The listing builds one solid part. Answer for the finished solid, in the listing's coordinates (mm). Face numbers are marked on the shaded views. Give positions to 0.01 mm unless a question says otherwise; leave off trailing zeros. Write each loop counter-clockwise with the first axis right and the second up, starting at its lowest first coordinate (ties: lowest second). Pieces come first, ordered by that corner, then holes.
```python
from build123d import *

# Parameters (mm, degrees)
SKETCH_1_R      = 5.1
EXTRUDE_1_DEPTH = 12


with BuildPart() as part:
    # 草图1 → 凸台-拉伸1 (new, symmetric)
    with BuildSketch(Plane.XY):
        with BuildLine():
            Line((0, 15), (30, 15))
            Line((30, 15), (30, -15))
            Line((30, -15), (0, -15))
            ThreePointArc((0, -15), (-15, 0), (0, 15))
        make_face()
        Circle(SKETCH_1_R, mode=Mode.SUBTRACT)
    extrude(amount=EXTRUDE_1_DEPTH, both=True)


solid = part.part
```
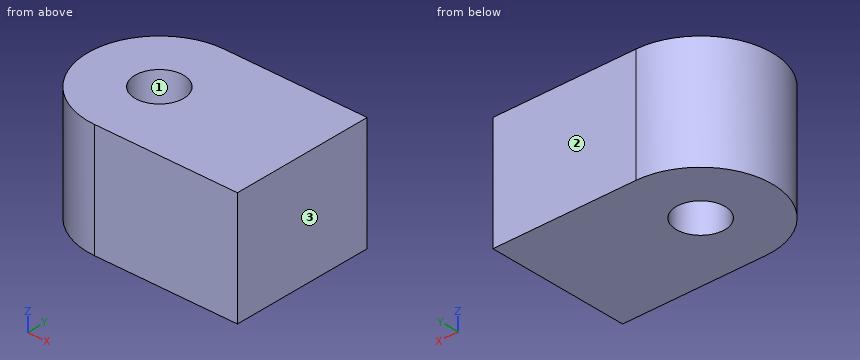
Item 1: A cutting plane is placed at B-B, the plane y = 0. Give the vertices of the cut face in (x, z).
Conclusion:
outline: (-15, -12) - (-5.1, -12) - (-5.1, 12) - (-15, 12) - close; (5.1, -12) - (30, -12) - (30, 12) - (5.1, 12) - close
Item 2: Each of these flat-tipped pins is pushed along its axis until it touches: P1, Ø12, axis at x = -4, z = -8, coming from the +Y side; P2, Ø10, axis at x = -6.5, z = 2, coming from the -Y side. Where does it stop, or does it pass through?
Conclusion:
P1: stops at y = 15
P2: stops at y = -14.92
Item 3: A cutting plane is placed at D-D, the plane y = 5.75. Give the vertices of the cut face in (x, z).
Conclusion:
outline: (-13.85, -12) - (30, -12) - (30, 12) - (-13.85, 12) - close
Item 4: A cutting plane is placed at A-A, the plane z = -1.25. Give the vertices of the cut face in (x, y).
Conclusion:
outline: (0, -15) - (30, -15) - (30, 15) - (0, 15) arc R15 ccw to start; hole circle Ø10.2 at (0, 0)
Item 5: Determine the mould class of the marked faces 1, 2 and 3 for opening direction X: pulls with the +X half, pulls with the -X half, needs draft (parallel to the pull), parting line crosses it, or undercut.
Conclusion:
face 1: undercut
face 2: needs draft
face 3: pulls with the +X half
Item 6: Consider probe 1 along Y at (x, z) = (0, -4.25); probe 2 along X at (y, z) = (3, -1.5); probe 3 along X at (y, z) = (-0.5, -1.25). Determine where each line is inside the solid, lowest interval first.
Conclusion:
probe 1: y = -15 to -5.1, 5.1 to 15
probe 2: x = -14.7 to -4.12, 4.12 to 30
probe 3: x = -14.99 to -5.08, 5.08 to 30
Item 7: A cutting plane is placed at C-C, the plane x = -8.5. Give the vertices of the cut face in (y, z), plus the area to 3 significant figures.
Conclusion:
outline: (-12.36, -12) - (12.36, -12) - (12.36, 12) - (-12.36, 12) - close
area: 593 mm2
